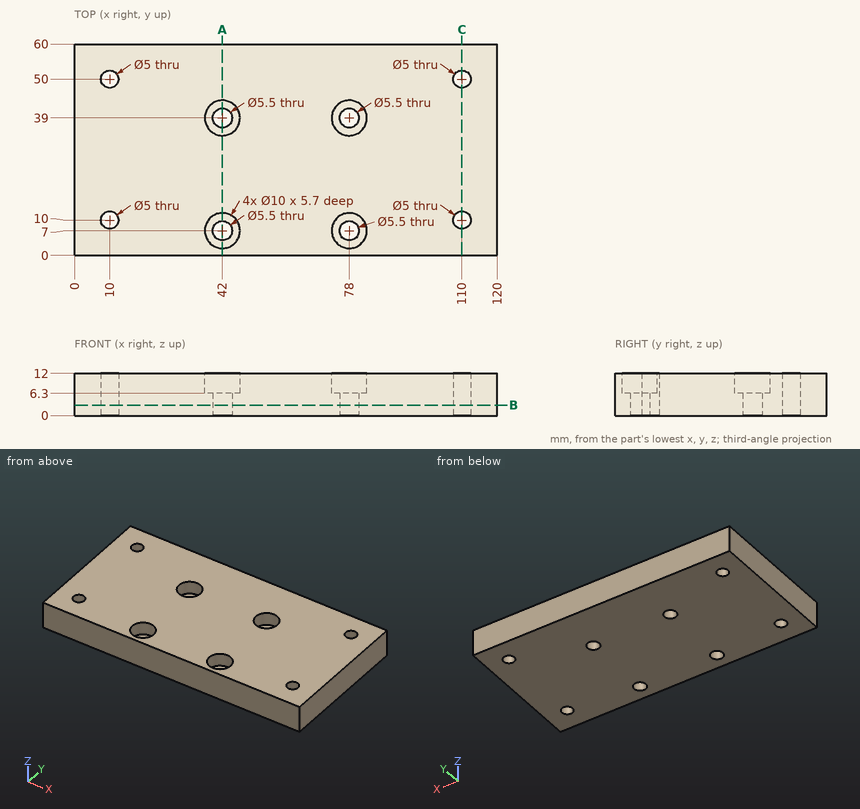
The drawing under review shows one solid part. Ordinate dimensions are in mm from its lowest x, y, z. Give positions to 0.01 mm unless a question says otherwise; leave off trailing zeros. Loops run counter-clockwise (first coordinate to the right, second up) from the corner with the lowest first, then second, coordinate; pieces in that order, holes last. Notation, with made-up numbers: M 74,-37 L 99,-37 A32 ccw 99,-1 Z; hole C 61,7 d7. An arc over 180 degrees is marked long. Return JSON: item names as keys, results as strings. Group by question number.
Item 1: For probe 1 along Y at (x, z) = (78, 8.6); probe 2 along Y at (x, z) = (10, 5.25); probe 3 along Z at (x, y) = (75, 42.5), list the stretches that pass through material, from the lowest coordinate up.
Item 2: Insertion check: pin 1 Ø4 at (x, y) = (110, 10) entering from +Z; pin 2 Ø5 at (x, y) = (44, 6.5) entering from +Z. Each pin has a flat end and moves straight along its axis. Give the tip position at first contact, or say it passes through.
Item 3: We need section A-A (x = 42). Give the boundary of the cut face in (y, z).
Item 4: We need section B-B (z = 3). Give the number of separate pieces and of enclosed holes in the cut face, and give its area (3 significant figures).
Item 5: We need section C-C (x = 110). Give the boundary of the cut face in (y, z).
Output:
{
 "1": {"probe 1": "y = 0 to 2, 12 to 34, 44 to 60", "probe 2": "y = 0 to 7.5, 12.5 to 47.5, 52.5 to 60", "probe 3": "z = 0 to 6.3"},
 "2": {"pin 1": "passes through", "pin 2": "stops at z = 6.3"},
 "3": {"outline": "M 0,0 L 4.25,0 L 4.25,6.3 L 2,6.3 L 2,12 L 0,12 Z; M 9.75,0 L 36.25,0 L 36.25,6.3 L 34,6.3 L 34,12 L 12,12 L 12,6.3 L 9.75,6.3 Z; M 41.75,0 L 60,0 L 60,12 L 44,12 L 44,6.3 L 41.75,6.3 Z"},
 "4": {"separate pieces": "1", "enclosed holes": "8", "area": "7,030 mm^2"},
 "5": {"outline": "M 0,0 L 7.5,0 L 7.5,12 L 0,12 Z; M 12.5,0 L 47.5,0 L 47.5,12 L 12.5,12 Z; M 52.5,0 L 60,0 L 60,12 L 52.5,12 Z"}
}
